from build123d import *

# Parameters (mm, degrees)
SKETCH1_W           = 57
SKETCH1_H           = 57
BOSS_EXTRUDE1_DEPTH = 56
SKETCH2_R           = 2.5
CUT_EXTRUDE1_DEPTH  = 98
SKETCH4_R           = 10
BOSS_EXTRUDE2_DEPTH = 1
SKETCH5_R           = 4
BOSS_EXTRUDE3_DEPTH = 21
CUT_EXTRUDE2_DEPTH  = 21
SKETCH7_R           = 12.5
CUT_EXTRUDE3_DEPTH  = 46


with BuildPart() as part:
    # Sketch1 → Boss-Extrude1 (new body)
    with BuildSketch(Plane.XY):
        Rectangle(SKETCH1_W, SKETCH1_H)
    extrude(amount=BOSS_EXTRUDE1_DEPTH)

    # Sketch2 → Cut-Extrude1 (cut)
    with BuildSketch(Plane.XY.offset(56)):
        with Locations((-23.5, 23.5)):
            Circle(SKETCH2_R)
        with Locations((23.5, 23.5)):
            Circle(SKETCH2_R)
        with Locations((23.5, -23.5)):
            Circle(SKETCH2_R)
        with Locations((-23.5, -23.5)):
            Circle(SKETCH2_R)
    extrude(amount=-CUT_EXTRUDE1_DEPTH, mode=Mode.SUBTRACT)

    # Sketch4 → Boss-Extrude2 (add)
    with BuildSketch(Plane.XY.offset(56)):
        Circle(SKETCH4_R)
    extrude(amount=BOSS_EXTRUDE2_DEPTH)

    # Sketch5 → Boss-Extrude3 (add)
    with BuildSketch(Plane.XY.offset(57)):
        with Locations(Location((0, 0, 0), (0, 0, 180))):
            Circle(SKETCH5_R)
    extrude(amount=BOSS_EXTRUDE3_DEPTH)

    # Sketch6 → Cut-Extrude2 (cut)
    with BuildSketch(Plane.XY.offset(78)):
        Polygon((3, 101.241638907), (3, 2.645751311), (3, -2.645751311), (3, -101.241638907), (200.191775192, -101.241638907), (200.191775192, 101.241638907), align=None)
    extrude(amount=-CUT_EXTRUDE2_DEPTH, mode=Mode.SUBTRACT)

    # Sketch7 → Cut-Extrude3 (cut)
    with BuildSketch(Plane(origin=(0, 0, 0), x_dir=(-1, 0, 0), z_dir=(0, 0, -1))):
        with Locations((-28.5, 28.5)):
            Circle(SKETCH7_R)
        with Locations((28.5, 28.5)):
            Circle(SKETCH7_R)
        with Locations((28.5, -28.5)):
            Circle(SKETCH7_R)
        with Locations((-28.5, -28.5)):
            Circle(SKETCH7_R)
    extrude(amount=-CUT_EXTRUDE3_DEPTH, mode=Mode.SUBTRACT)


solid = part.part
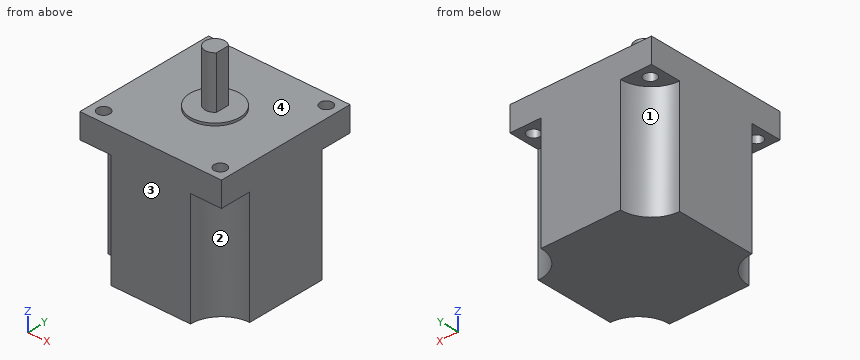
Can you work these out from the model? Positions are in its coordinate system, mm. Face numbers are marked on the shaded views. A direction names the side the tool comes from. Round coordinates to 2 decimals unless told otherwise and drop trailing zeros. Loops run counter-clockwise (first coordinate to the right, second up) from the corner with the lowest first, then second, coordinate; pieces in that order, holes last. Notation, with made-up numbers: (37, 4) - (87, 4) arc R17 cw to (87, 8) - close; hole circle Ø6 at (-38.5, 3.5). An arc over 180 degrees is marked (long way). Use CSV: the item, a comma, the result in double quotes. Start each with the question number.
1) If we section it at A-A on x = 25: Write out the boundary of the cut face in (y, z), plus the area to 3 significant figures.
2) Please list where these lines run through material, in increasing order: probe 1 along Y at (x, z) = (23.5, 53.5); probe 2 along Z at (x, y) = (20.5, 0); probe 3 along Z at (x, y) = (-3.5, -6.5). Write a range as [from, to].
3) If we section it at B-B on z = 12: Write out the boundary of the cut face in (x, y).
4) If we section it at D-D on x = 0: Write out the boundary of the cut face in (y, z), plus the area to 3 significant figures.
5) For pin 1 Ø10 at (x, y) = (25.5, 23.5) entering from -Z; pin 2 Ø5 at (x, y) = (-21, 14.5) entering from +Z; pin 3 Ø6 at (y, z) = (0.5, 70) entering from +X, each with a flat end and sliding along its axis, tell me the tip position at first contact or that it passes through.
6) If we section it at C-C on y = 23.5: Write out the boundary of the cut face in (x, z).
7) For the marked faces 1, 2, 3 and 4, which set-ups out of +Z, -Z, +X, -X, +Y, -Y let a thin tool reach every point of the face, with its end or its side?
Geometry results:
1,outline,"(-28.5, 46) - (-25.5, 46) - (-25.5, 56) - (-28.5, 56) - close; (-21.5, 46) - (-16.5, 46) - (-16.5, 0) - (16.5, 0) - (16.5, 46) - (21.5, 46) - (21.5, 56) - (-21.5, 56) - close; (25.5, 46) - (28.5, 46) - (28.5, 56) - (25.5, 56) - close"
1,area,"2,010 mm2"
2,probe 1,"y = [-28.5, -26], [-21, 21], [26, 28.5]"
2,probe 2,"z = [0, 56]"
2,probe 3,"z = [0, 57]"
3,outline,"(-28.5, -16) arc R12.5 cw to (-16, -28.5) - (16, -28.5) arc R12.5 cw to (28.5, -16) - (28.5, 16) arc R12.5 cw to (16, 28.5) - (-16, 28.5) arc R12.5 cw to (-28.5, 16) - close"
4,outline,"(-28.5, 0) - (28.5, 0) - (28.5, 56) - (10, 56) - (10, 57) - (4, 57) - (4, 78) - (-4, 78) - (-4, 57) - (-10, 57) - (-10, 56) - (-28.5, 56) - close"
4,area,"3,380 mm2"
5,pin 1,"stops at z = 46"
5,pin 2,"stops at z = 56"
5,pin 3,"stops at x = 3"
6,outline,"(-28.5, 46) - (-26, 46) - (-26, 56) - (-28.5, 56) - close; (-21, 46) - (-17.04, 46) - (-17.04, 0) - (17.04, 0) - (17.04, 46) - (21, 46) - (21, 56) - (-21, 56) - close; (26, 46) - (28.5, 46) - (28.5, 56) - (26, 56) - close"
7,face 1,"-Z, -X, +Y"
7,face 2,"-Z, +X, -Y"
7,face 3,"+Z, -Z, +X, -X, -Y"
7,face 4,"+Z"
